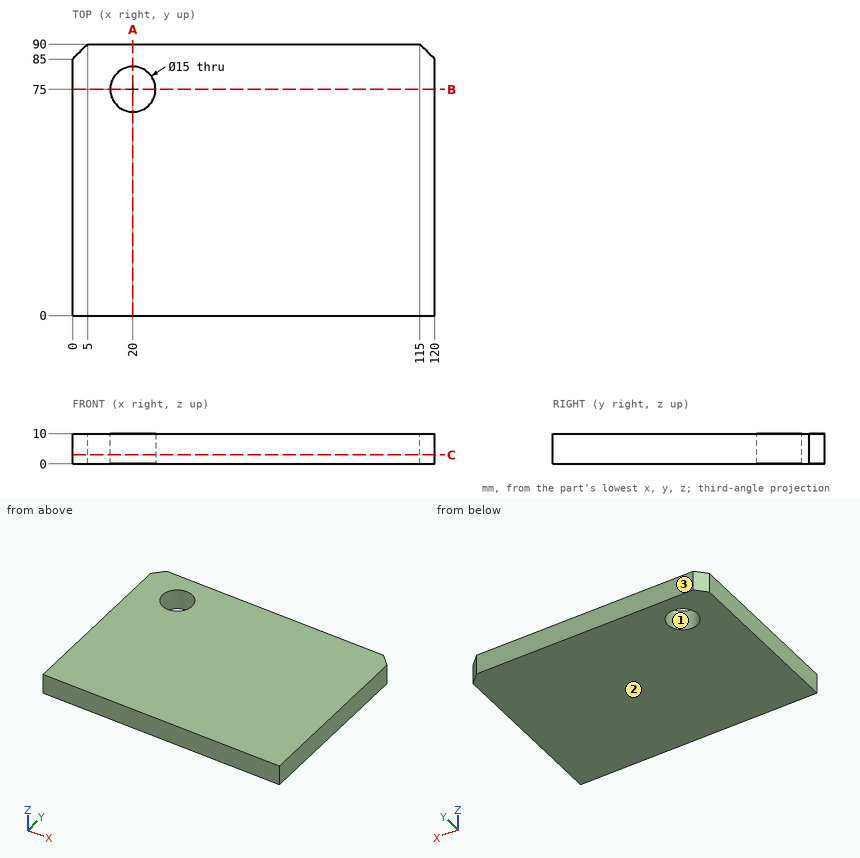
Verification items for this drawing (mm, ordinates from the low corner). Coordinates: 2 decimals unless noted, no trailing zeros. Order: outer loops, then holes, each group sorted by start corner. A loop starts at its lowest first (then second) coordinate and runs counter-clockwise, first axis right, second up. Notation, with made-up numbers: (-28.75, 55.25) - (22.25, 55.25) arc R12 cw to (22.25, 70.25) - close; hole circle Ø10 at (23, -38). An arc over 180 degrees is marked (long way). Answer as a JSON object with one key per item and string values. Group by question number.
Item 1: Sectioned sample at C-C, the plane z = 3. Record the cut outline in (x, y).
Item 2: Scan lines: probe 1 along Y at (x, z) = (20, 5.25); probe 2 along X at (y, z) = (71.5, 6.75); probe 3 along X at (y, z) = (79, 9.75). Record each from-to range of solid material in increasing order.
Item 3: Draft check along Y on the marked faces 1, 2 and 3. Enter one of: +Y half, -Y half, draft (parallel to the pull), parting line (faces both ways), or undercut.
Item 4: Sectioned sample at B-B, the plane y = 75. Record the cut outline in (x, z).
Item 5: Sectioned sample at A-A, the plane x = 20. Record the cut outline in (y, z).
Resolved:
{
 "1": {"outline": "(0, 0) - (120, 0) - (120, 85) - (115, 90) - (5, 90) - (0, 85) - close; hole circle Ø15 at (20, 75)"},
 "2": {"probe 1": "0 to 67.5, 82.5 to 90", "probe 2": "0 to 13.37, 26.63 to 120", "probe 3": "0 to 13.66, 26.34 to 120"},
 "3": {"face 1": "undercut", "face 2": "draft", "face 3": "+Y half"},
 "4": {"outline": "(0, 0) - (12.5, 0) - (12.5, 10) - (0, 10) - close; (27.5, 0) - (120, 0) - (120, 10) - (27.5, 10) - close"},
 "5": {"outline": "(0, 0) - (67.5, 0) - (67.5, 10) - (0, 10) - close; (82.5, 0) - (90, 0) - (90, 10) - (82.5, 10) - close"}
}
